Check sheet for the modelled part. Datum: model origin and axes. Units: mm. A direction names the side the tool comes from. Give positions to 0.01 mm unless a question says otherwise; leave off trailing zeros. Write each loop counter-clockwise with the first axis right and the second up, starting at its lowest first coordinate (ties: lowest second). Pieces come first, ordered by that corner, then holes. Notation, with made-up numbers: (70.5, 55.5) -> (115.5, 55.5) arc R22 cw to (115.5, 66.5) -> close; hole circle Ø11 at (14, 55). An arc over 180 degrees is marked (long way). Use a Markdown table: item, result. Add a question column.
1. Cross-section at B-B (z = 65.5). Enter the section's corners in (x, y), then the cut area to 4 significant figures.
2. Release check for a two-part mould opening along X. For faces 1 (the flat face through (-107, 0, 101)), 2 (the cylindrical face through (-35.87, 9.86, -64.31)), 3 (the flat face through (-114, 10, 21)) record: released by +X, released by -X, zero draft, split by the parting line, or undercut.
3. Scan lines: probe 1 along Z at (x, y) = (-226, 19.25); probe 2 along X at (y, z) = (2, 90.5); probe 3 along Z at (x, y) = (-193, 2). Record each from-to range of solid material in increasing order. Write a range as [from, to].
4. Cross-section at D-D (x = -20). Enter the section's corners in (y, z), then the cut area to 3 significant figures.
5. Set-up check for faces 4 (the cylindrical face through (-146.473, 15.07, 50.856)), 5 (the flat face through (-112, 10, 193)), 6 (the flat face through (-229, 10, 42.659)), 7 (the flat face through (-107, 20, 108)): record each of +Z, -Z, +X, -X, +Y, -Y from which the full face is reachable in a straight line by a thin tool's end or side.
6. Cross-section at C-C (x = -180). Enter the section's corners in (y, z), then the cut area to 3 significant figures.
7. Cross-section at A-A (x = -240). Enter the section's corners in (y, z).
8. Gauge pin test, flat ends, axial feed: P1, Ø1.5, axis at y = 5.5, z = 177, coming from the +X side; P2, Ø4, axis at y = 2, z = 90, coming from the -X side; P3, Ø2.5, axis at x = -240.5, y = 2.5, coming from the -Z side; P4, Ø5, axis at x = -175.5, y = 9, coming from the -Z side. Record the tip position at first contact, or that the pin passes through.
from build123d import *

# Parameters (mm, degrees)
EXTRUDE_1_DEPTH      = 20
CUT_EXTRUDE_1_DEPTH  = 10
SKETCH_4_W           = 45
SKETCH_4_H           = 90
CUT_EXTRUDE_2_DEPTH  = 5
SKETCH_5_W           = 112
SKETCH_5_H           = 20
EXTRUDE_2_DEPTH      = 40
CUT_EXTRUDE_3_REACH  = 1227.871
SKETCH_6_R           = 6
SKETCH_6_R_2         = 5
CUT_EXTRUDE_4_REACH  = 1228.116
SKETCH_7_R           = 7.332886018
SKETCH_7_R_2         = 7.301331484
SKETCH_7_R_3         = 6.603217824
SKETCH_24_R          = 6
CUT_EXTRUDE_21_DEPTH = 25


with BuildPart() as part:
    # 草图1 → 凸台-拉伸1 (new body)
    with BuildSketch(Plane(origin=(0, 0, 0), x_dir=(1, 0, 0), z_dir=(0, 1, 0))):
        with BuildLine():
            Line((-190, -173.659488393), (0, -173.659488393))
            Line((0, -173.659488393), (0, 71.340511607))
            ThreePointArc((0, 71.340511607), (-36.354926075, 64.109067196), (-67.175144213, 43.51565582))
            add(Edge.make_bspline(
                [(-122.824855787, -14.834632605), (-95, 14.340511607), (-67.175144213, 43.51565582)],
                knots=[0, 0, 0, 1, 1, 1], degree=2))
            ThreePointArc((-122.824855787, -14.834632605), (-153.645073925, -35.428043981), (-190, -42.659488393))
            Line((-190, -42.659488393), (-270, -42.659488393))
            Line((-270, -42.659488393), (-270, -173.659488393))
            Line((-270, -173.659488393), (-190, -173.659488393))
        make_face()
    extrude(amount=EXTRUDE_1_DEPTH)

    # 草图2 → 切除-拉伸1 (cut)
    with BuildSketch(Plane(origin=(0, 20, 0), x_dir=(1, 0, 0), z_dir=(0, 1, 0))):
        with BuildLine():
            Line((-270, -52.659488393), (-190, -52.659488393))
            ThreePointArc((-190, -52.659488393), (-149.762170559, -44.64359576), (-115.668000558, -21.819813762))
            Line((-115.668000558, -21.819813762), (-60.022606457, 36.52594767))
            ThreePointArc((-60.022606457, 36.52594767), (-32.474897495, 54.892284551), (0, 61.340511607))
            Line((0, 61.340511607), (0, 54.340511607))
            ThreePointArc((0, 54.340511607), (-29.760862596, 48.439686759), (-55.01881141, 31.630025903))
            Line((-55.01881141, 31.630025903), (-110.655962205, -26.707092192))
            ThreePointArc((-110.655962205, -26.707092192), (-147.042646878, -51.093843482), (-190, -59.659488393))
            Line((-190, -59.659488393), (-270, -59.659488393))
            Line((-270, -59.659488393), (-270, -52.659488393))
        make_face()
    extrude(amount=-CUT_EXTRUDE_1_DEPTH, mode=Mode.SUBTRACT)

    # 草图4 → 切除-拉伸2 (cut)
    with BuildSketch(Plane.XZ):
        with Locations((-247.5, 99.659488393)):
            Rectangle(SKETCH_4_W, SKETCH_4_H)
    extrude(amount=-CUT_EXTRUDE_2_DEPTH, mode=Mode.SUBTRACT)

    # 草图5 → 凸台-拉伸2 (add)
    with BuildSketch(Plane.XY.offset(173.659488393)):
        with Locations((-56, 10)):
            Rectangle(SKETCH_5_W, SKETCH_5_H)
    extrude(amount=EXTRUDE_2_DEPTH)

    # 切除-拉伸3: up to this face of the body (flat: up to its plane)
    cut_extrude_3_end = Plane(part.part.faces().sort_by_distance((-99.039367246, 0, 91.650022184))[0])
    # 草图6 → 切除-拉伸3 (cut, up to the picked face)
    with BuildSketch(Plane(origin=(600.126281628, 25, -649.482989384), x_dir=(0, 0, -1), z_dir=(0, 1, 0)), mode=Mode.PRIVATE) as cut_extrude_3_sk1:
        with Locations(Location((-666.704267343, 635.126281628, 0), (0, 0, 180))):
            Circle(SKETCH_6_R)
    cut_extrude_3_tool1 = split(extrude(cut_extrude_3_sk1.sketch, amount=-CUT_EXTRUDE_3_REACH, mode=Mode.PRIVATE), bisect_by=cut_extrude_3_end, keep=Keep.BOTH, mode=Mode.PRIVATE)
    # 草图6 → 切除-拉伸3 (cut, up to the picked face)
    with BuildSketch(Plane(origin=(600.126281628, 25, -649.482989384), x_dir=(0, 0, -1), z_dir=(0, 1, 0)), mode=Mode.PRIVATE) as cut_extrude_3_sk2:
        with Locations(Location((-746.704267343, 635.126281628, 0), (0, 0, 180))):
            Circle(SKETCH_6_R_2)
    cut_extrude_3_tool2 = split(extrude(cut_extrude_3_sk2.sketch, amount=-CUT_EXTRUDE_3_REACH, mode=Mode.PRIVATE), bisect_by=cut_extrude_3_end, keep=Keep.BOTH, mode=Mode.PRIVATE)
    # 草图6 → 切除-拉伸3 (cut, up to the picked face)
    with BuildSketch(Plane(origin=(600.126281628, 25, -649.482989384), x_dir=(0, 0, -1), z_dir=(0, 1, 0)), mode=Mode.PRIVATE) as cut_extrude_3_sk3:
        with Locations(Location((-746.704267343, 840.126281628, 0), (0, 0, 180))):
            Circle(SKETCH_6_R)
    cut_extrude_3_tool3 = split(extrude(cut_extrude_3_sk3.sketch, amount=-CUT_EXTRUDE_3_REACH, mode=Mode.PRIVATE), bisect_by=cut_extrude_3_end, keep=Keep.BOTH, mode=Mode.PRIVATE)
    # 草图6 → 切除-拉伸3 (cut, up to the picked face)
    with BuildSketch(Plane(origin=(600.126281628, 25, -649.482989384), x_dir=(0, 0, -1), z_dir=(0, 1, 0)), mode=Mode.PRIVATE) as cut_extrude_3_sk4:
        with Locations(Location((-746.704267343, 735.126281628, 0), (0, 0, 180))):
            Circle(SKETCH_6_R)
    cut_extrude_3_tool4 = split(extrude(cut_extrude_3_sk4.sketch, amount=-CUT_EXTRUDE_3_REACH, mode=Mode.PRIVATE), bisect_by=cut_extrude_3_end, keep=Keep.BOTH, mode=Mode.PRIVATE)
    add(cut_extrude_3_tool1.solids().sort_by(Axis((-35, 25, 17.221278), (0, -1, 0)))[0], mode=Mode.SUBTRACT)
    add(cut_extrude_3_tool2.solids().sort_by(Axis((-35, 25, 97.221278), (0, -1, 0)))[0], mode=Mode.SUBTRACT)
    add(cut_extrude_3_tool3.solids().sort_by(Axis((-240, 25, 97.221278), (0, -1, 0)))[0], mode=Mode.SUBTRACT)
    add(cut_extrude_3_tool4.solids().sort_by(Axis((-135, 25, 97.221278), (0, -1, 0)))[0], mode=Mode.SUBTRACT)

    # 草图7 → 切除-拉伸4 (cut, up to next)
    with BuildSketch(Plane(origin=(600.126281628, 35, -649.482989384), x_dir=(0, 0, -1), z_dir=(0, 1, 0)), mode=Mode.PRIVATE) as cut_extrude_4_sk1:
        with Locations(Location((-804.642477777, 640.126281628, 0), (0, 0, 180))):
            Circle(SKETCH_7_R)
    cut_extrude_4_tool1 = extrude(cut_extrude_4_sk1.sketch, amount=-CUT_EXTRUDE_4_REACH, mode=Mode.PRIVATE) & part.part
    # 草图7 → 切除-拉伸4 (cut, up to next)
    with BuildSketch(Plane(origin=(600.126281628, 35, -649.482989384), x_dir=(0, 0, -1), z_dir=(0, 1, 0)), mode=Mode.PRIVATE) as cut_extrude_4_sk2:
        with Locations(Location((-804.642477777, 710.126281628, 0), (0, 0, 180))):
            Circle(SKETCH_7_R_2)
    cut_extrude_4_tool2 = extrude(cut_extrude_4_sk2.sketch, amount=-CUT_EXTRUDE_4_REACH, mode=Mode.PRIVATE) & part.part
    # 草图7 → 切除-拉伸4 (cut, up to next)
    with BuildSketch(Plane(origin=(600.126281628, 35, -649.482989384), x_dir=(0, 0, -1), z_dir=(0, 1, 0)), mode=Mode.PRIVATE) as cut_extrude_4_sk3:
        with Locations(Location((-804.642477777, 780.126281628, 0), (0, 0, 180))):
            Circle(SKETCH_7_R_3)
    cut_extrude_4_tool3 = extrude(cut_extrude_4_sk3.sketch, amount=-CUT_EXTRUDE_4_REACH, mode=Mode.PRIVATE) & part.part
    add(cut_extrude_4_tool1.solids().sort_by_distance((-40, 35, 155.159488))[0], mode=Mode.SUBTRACT)
    add(cut_extrude_4_tool2.solids().sort_by_distance((-110, 35, 155.159488))[0], mode=Mode.SUBTRACT)
    add(cut_extrude_4_tool3.solids().sort_by_distance((-180, 35, 155.159488))[0], mode=Mode.SUBTRACT)

    # 草图24 → 切除-拉伸21 (cut)
    with BuildSketch(Plane(origin=(600.126281628, 25, -649.482989384), x_dir=(0, 0, -1), z_dir=(0, 1, 0))):
        with Locations(Location((-666.704267343, 635.126281628, 0), (0, 0, 180))):
            Circle(SKETCH_24_R)
        with Locations(Location((-746.704267343, 635.126281628, 0), (0, 0, 180))):
            Circle(SKETCH_24_R)
        with Locations(Location((-746.704267343, 840.126281628, 0), (0, 0, 180))):
            Circle(SKETCH_24_R)
        with Locations(Location((-746.704267343, 735.126281628, 0), (0, 0, 180))):
            Circle(SKETCH_24_R)
    extrude(amount=-CUT_EXTRUDE_21_DEPTH, mode=Mode.SUBTRACT)


solid = part.part
Worked answers:
| question | item | result |
|---|---|---|
| 1 | outline | (-270, 5) -> (-225, 5) -> (-225, 0) -> (0, 0) -> (0, 20) -> (-270, 20) -> close |
| 1 | area | 5,175 mm² |
| 2 | face 1 | zero draft |
| 2 | face 2 | released by -X |
| 2 | face 3 | undercut |
| 3 | probe 1 | z = [42.66, 52.66], [59.66, 173.66] |
| 3 | probe 2 | x = [-225, 0] |
| 3 | probe 3 | z = [42.66, 173.66] |
| 4 | outline | (0, -69.21) -> (20, -69.21) -> (20, -58.95) -> (10, -58.95) -> (10, -51.73) -> (20, -51.73) -> (20, 213.66) -> (0, 213.66) -> close |
| 4 | area | 5,590 mm² |
| 5 | face 4 | +Y |
| 5 | face 5 | +Z, -X, +Y, -Y |
| 5 | face 6 | -Z, -X, +Y, -Y |
| 5 | face 7 | +Z, -Z, +X, -X, +Y |
| 6 | outline | (0, 42.13) -> (20, 42.13) -> (20, 52.18) -> (10, 52.18) -> (10, 59.21) -> (20, 59.21) -> (20, 148.56) -> (0, 148.56) -> close; (0, 161.76) -> (20, 161.76) -> (20, 173.66) -> (0, 173.66) -> close |
| 6 | area | 2,300 mm² |
| 7 | outline | (0, 42.66) -> (20, 42.66) -> (20, 52.66) -> (10, 52.66) -> (10, 59.66) -> (20, 59.66) -> (20, 91.22) -> (5, 91.22) -> (5, 54.66) -> (0, 54.66) -> close; (0, 144.66) -> (5, 144.66) -> (5, 103.22) -> (20, 103.22) -> (20, 173.66) -> (0, 173.66) -> close |
| 8 | P1 | stops at x = 0 |
| 8 | P2 | stops at x = -225 |
| 8 | P3 | stops at z = 42.66 |
| 8 | P4 | stops at z = 41.13 |
